from build123d import *

# Parameters (mm, degrees)
SKETCH_1_W      = 660
SKETCH_1_H      = 300
EXTRUDE_1_DEPTH = 500
SHELL_1_T       = -10


with BuildPart() as part:
    # 草图1 → 凸台-拉伸1 (new body)
    with BuildSketch(Plane.XY):
        with Locations((-674.904398529, 2868.914811934)):
            Rectangle(SKETCH_1_W, SKETCH_1_H)
    extrude(amount=EXTRUDE_1_DEPTH)

    # 抽壳1
    shell_1_openings = [part.faces().sort_by_distance(p)[0] for p in [
        (-674.904398529, 2868.914811934, 0),
    ]]
    offset(amount=SHELL_1_T, openings=shell_1_openings, kind=Kind.INTERSECTION)


solid = part.part
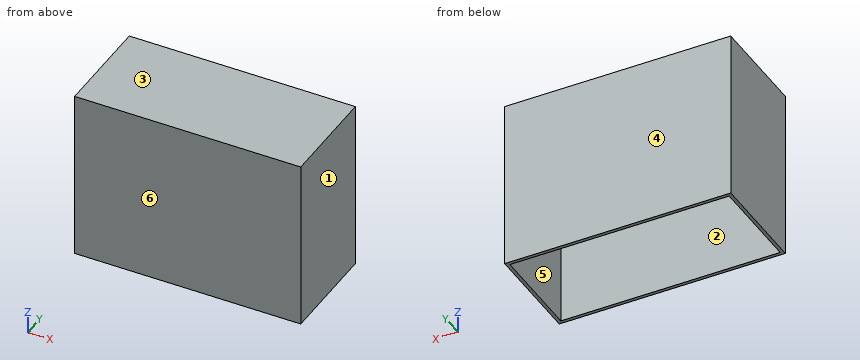
Could you check a few things on this model? Use its own coordinates, in mm. Face numbers are marked on the shaded views. A direction names the side the tool comes from. Coordinates: 2 decimals unless noted, no trailing zeros. Write each loop counter-clockwise with the first axis right and the second up, starting at its lowest first coordinate (ties: lowest second). Pieces come first, ordered by that corner, then holes. Notation, with made-up numbers: (-10, -35.5) - (12, -35.5) arc R29 cw to (12, 0.5) - close; hole circle Ø8 at (77.5, 66). An arc over 180 degrees is marked (long way). Write item = value, one per line.
1) Suppose I cut it at B-B on x = -407.5. Please give me the cut outline in (y, z), plus the area to 3 significant figures.
Result set:
outline = (2718.91, 0) - (2728.91, 0) - (2728.91, 490) - (3008.91, 490) - (3008.91, 0) - (3018.91, 0) - (3018.91, 500) - (2718.91, 500) - close
area = 12,800 mm2
2) For the marked faces 1 and 2, which set-ups out of +Z, -Z, +X, -X, +Y, -Y let a thin tool reach every point of the face, with its end or its side?
Result set:
face_1 = +Z, -Z, +X, +Y, -Y
face_2 = -Z
3) Suppose I cut it at A-A on z = 340. Please give me the cut outline in (x, y).
Result set:
outline = (-1004.9, 2718.91) - (-344.9, 2718.91) - (-344.9, 3018.91) - (-1004.9, 3018.91) - close; hole (-994.9, 2728.91) - (-354.9, 2728.91) - (-354.9, 3008.91) - (-994.9, 3008.91) - close
4) Suppose I cut it at C-C on y = 3001. Please give me the cut outline in (x, z).
Result set:
outline = (-1004.9, 0) - (-994.9, 0) - (-994.9, 490) - (-354.9, 490) - (-354.9, 0) - (-344.9, 0) - (-344.9, 500) - (-1004.9, 500) - close
5) Will this pin go through, and if not, where does the flat tip stop? pin 1 Ø4 at (x, y) = (-573.5, 2838.5) entering from -Z.
Result set:
pin_1 = 490
6) We'd pull the mould along Y, two halves only. Please class the marked faces 3, 4, 5 and 6: +Y half, -Y half, draft (parallel to the pull), parting line (faces both ways), or undercut.
Result set:
face_3 = draft
face_4 = +Y half
face_5 = undercut
face_6 = -Y half
7) Please list where these lines run through material, in increasing order: line 1 (Y direction, x = -596, z = 385); line 2 (X direction, y = 2960, z = 322.5); line 3 (Z direction, x = -852, y = 2808.5). Write a range as [from, to].
Result set:
line_1 = [2718.91, 2728.91], [3008.91, 3018.91]
line_2 = [-1004.9, -994.9], [-354.9, -344.9]
line_3 = [490, 500]
